```python
from build123d import *

# Parameters (mm, degrees)
SKETCH_1_R      = 1.525
SKETCH_1_W      = 41.5
SKETCH_1_H      = 21.5
SKETCH_1_W_2    = 10
SKETCH_1_H_2    = 3
EXTRUDE_3_DEPTH = 3


with BuildPart() as part:
    # 草图1 → 凸台-拉伸3 (new body)
    with BuildSketch(Plane.XY):
        Polygon((-77.274452038, 15.659691017), (-82.274452038, 10.659691017), (-82.274452038, -10.840308983), (-77.274452038, -15.840308983), (-24.774452038, -15.840308983), (-14.844452038, -10.090308983), (15.155547962, -10.090308983), (25.085547962, -15.840308983), (77.585547962, -15.840308983), (82.585547962, -10.840308983), (82.585547962, 10.659691017), (77.585547962, 15.659691017), (25.085547962, 15.659691017), (15.155547962, 9.909691017), (-14.844452038, 9.909691017), (-24.774452038, 15.659691017), align=None)
        with Locations((78.135547962, 4.784691017)):
            Circle(SKETCH_1_R, mode=Mode.SUBTRACT)
        with Locations((78.135547962, -4.965308983)):
            Circle(SKETCH_1_R, mode=Mode.SUBTRACT)
        with Locations((-77.824452038, -4.965308983)):
            Circle(SKETCH_1_R, mode=Mode.SUBTRACT)
        with Locations((-77.824452038, 4.784691017)):
            Circle(SKETCH_1_R, mode=Mode.SUBTRACT)
        with Locations((29.535547962, 4.784691017)):
            Circle(SKETCH_1_R, mode=Mode.SUBTRACT)
        with Locations((29.535547962, -4.965308983)):
            Circle(SKETCH_1_R, mode=Mode.SUBTRACT)
        with Locations((-29.224452038, -4.965308983)):
            Circle(SKETCH_1_R, mode=Mode.SUBTRACT)
        with Locations((-29.224452038, 4.784691017)):
            Circle(SKETCH_1_R, mode=Mode.SUBTRACT)
        with Locations((-53.524452038, -0.090308983)):
            Rectangle(SKETCH_1_W, SKETCH_1_H, mode=Mode.SUBTRACT)
        with Locations((53.835547962, -0.090308983)):
            Rectangle(SKETCH_1_W, SKETCH_1_H, mode=Mode.SUBTRACT)
        with Locations((15.403552423, -0.090308983)):
            Rectangle(SKETCH_1_W_2, SKETCH_1_H_2, mode=Mode.SUBTRACT)
        with Locations((-15.092456498, -0.090308983)):
            Rectangle(SKETCH_1_W_2, SKETCH_1_H_2, mode=Mode.SUBTRACT)
    extrude(amount=EXTRUDE_3_DEPTH)


solid = part.part
```
The model under review builds one solid part; all positions refer to its coordinate system, in mm. A direction names the side the tool comes from. Round coordinates to 2 decimals unless told otherwise and drop trailing zeros. Loops run counter-clockwise (first coordinate to the right, second up) from the corner with the lowest first, then second, coordinate; pieces in that order, holes last. Notation, with made-up numbers: (-24.5, -11) -> (30.5, -11) arc R28 ccw to (30.5, 22) -> close; hole circle Ø7 at (-15.75, -29). An arc over 180 degrees is marked (long way). Answer as a JSON object with one key per item and string values. Group by question number.
1) For pin 1 Ø0.9 at (x, z) = (16.5, 2) entering from +Y; pin 2 Ø1 at (x, z) = (-2, 0.5) entering from -Y; pin 3 Ø1.5 at (x, z) = (-16.5, 2) entering from -Y, all flat-tipped, find the tip position at first contact; note any pin that passes through.
2) For line 1 (X direction, y = -1.5, z = 0.85); line 2 (X direction, y = 6.5, z = 1.7); line 3 (Y direction, x = -52, z = 2.5), list the stretches that pass through material, from the lowest coordinate up. Write a range as [from, to].
3) Mouldability with a two-part tool opening along X and no side actions: class faces 5 (the face through (20.404, 0, 1)), 6 (the face through (80.051, -13.375, 1.479)), 7 (the face through (52, 15.66, 1)) as released by +X, released by -X, zero draft, split by the parting line, or undercut.
4) We need section B-B on x = -3. Write out the cut boundary in (y, z).
5) For faces 1 (the face through (74.586, 0, 1)), 2 (the face through (0, 9.91, 1)), 3 (the face through (0, -10.09, 1)), 4 (the face through (-79.739, 13.195, 1.479)), list the 3-axis set-ups (+Z, -Z, +X, -X, +Y, -Y) from which the entire face can be reached by the end or side of a thin tool; tool diameter is ignored.
6) We need section A-A on x = -43. Write out the cut boundary in (y, z), then the cut area to 3 significant figures.
7) We need section D-D on x = 23.5. Write out the cut boundary in (y, z), then the cut area to 3 significant figures.
8) We need section C-C on z = 1.1. Give the number of separate pieces and of enclosed holes in the cut face, then the cut area to 3 significant figures.
Result set:
{
 "1": {"pin 1": "y = 10.95", "pin 2": "y = -10.09", "pin 3": "y = -11.48"},
 "2": {"line 1": "[-82.27, -74.27], [-32.77, -20.09], [-10.09, 10.4], [20.4, 33.09], [74.59, 82.59]", "line 2": "[-82.27, -74.27], [-32.77, 33.09], [74.59, 82.59]", "line 3": "[-15.84, -10.84], [10.66, 15.66]"},
 "3": {"face 5": "undercut", "face 6": "released by +X", "face 7": "zero draft"},
 "4": {"outline": "(-10.09, 0) -> (9.91, 0) -> (9.91, 3) -> (-10.09, 3) -> close"},
 "5": {"face 1": "+Z, -Z", "face 2": "+Z, -Z, +Y", "face 3": "+Z, -Z, -Y", "face 4": "+Z, -Z, -X, +Y"},
 "6": {"outline": "(-15.84, 0) -> (-10.84, 0) -> (-10.84, 3) -> (-15.84, 3) -> close; (10.66, 0) -> (15.66, 0) -> (15.66, 3) -> (10.66, 3) -> close", "area": "30.0 mm²"},
 "7": {"outline": "(-14.92, 0) -> (14.74, 0) -> (14.74, 3) -> (-14.92, 3) -> close", "area": "89.0 mm²"},
 "8": {"separate pieces": "1", "enclosed holes": "12", "area": "2,780 mm²"}
}
